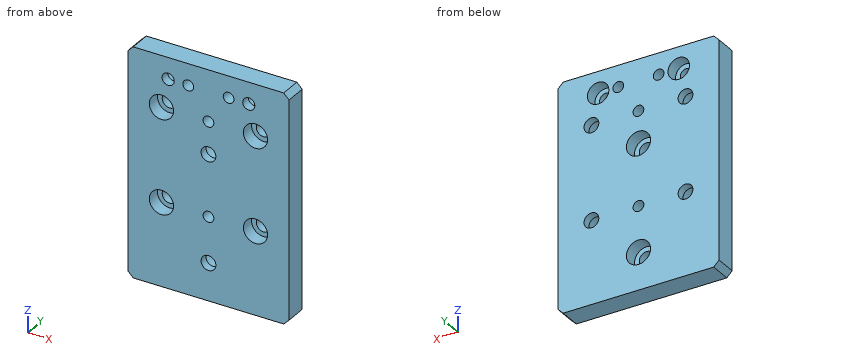
```python
from build123d import *

# Parameters (mm, degrees)
SKETCH_1_W                  = 60
SKETCH_1_H                  = 85
EXTRUDE_1_DEPTH             = 8
HOLE_WIZARD_1_D             = 5.5
HOLE_WIZARD_1_CBORE_D       = 9
HOLE_WIZARD_1_CBORE_DEPTH   = 5
HOLE_WIZARD_2_D             = 5.5
HOLE_WIZARD_2_DEPTH         = 12.4
HOLE_WIZARD_2_CBORE_D       = 9
HOLE_WIZARD_2_CBORE_DEPTH   = 5
HOLE_WIZARD_2_TIP           = 1.652366702
HOLE_WIZARD_1_2_D           = 4.5
HOLE_WIZARD_1_2_CBORE_D     = 8
HOLE_WIZARD_1_2_CBORE_DEPTH = 4.6
HOLE_WIZARD_4_0_4_1_D       = 4
CHAMFER_1_SIZE              = 2


with BuildPart() as part:
    # 草图1 → 凸台-拉伸1 (new body)
    with BuildSketch(Plane(origin=(0, 0, 0), x_dir=(1, 0, 0), z_dir=(0, 1, 0))):
        Rectangle(SKETCH_1_W, SKETCH_1_H)
    extrude(amount=EXTRUDE_1_DEPTH)

    # Hole Wizard 1 (through all)
    with Locations(Plane(origin=(0, 0, 0), x_dir=(-1, 0, 0), z_dir=(0, -1, 0))):
        with Locations((17.5, -23.45), (-17.5, -23.45), (17.5, 11.55), (-17.5, 11.55)):
            CounterBoreHole(HOLE_WIZARD_1_D / 2, HOLE_WIZARD_1_CBORE_D / 2, HOLE_WIZARD_1_CBORE_DEPTH)

    # 大小六角凹头盖螺钉柱孔2
    with Locations(Plane(origin=(0, 8, 0), x_dir=(1, 0, 0), z_dir=(0, 1, 0))):
        with Locations((0, 28.554479799), (0, -11.445520201)):
            CounterBoreHole(HOLE_WIZARD_2_D / 2, HOLE_WIZARD_2_CBORE_D / 2, HOLE_WIZARD_2_CBORE_DEPTH, depth=HOLE_WIZARD_2_DEPTH)
            with Locations((0, 0, -(HOLE_WIZARD_2_DEPTH + HOLE_WIZARD_2_TIP / 2))):  # 118° drill point
                Cone(0, HOLE_WIZARD_2_D / 2, HOLE_WIZARD_2_TIP, mode=Mode.SUBTRACT)

    # Hole Wizard 1 2 (through all)
    with Locations(Plane(origin=(0, 8, 0), x_dir=(1, 0, 0), z_dir=(0, 1, 0))):
        with Locations((-15, -34.5), (15, -34.5)):
            CounterBoreHole(HOLE_WIZARD_1_2_D / 2, HOLE_WIZARD_1_2_CBORE_D / 2, HOLE_WIZARD_1_2_CBORE_DEPTH)

    # Ø4.0 (4) 直径孔1 (through all)
    with Locations(Plane(origin=(0, 8, 0), x_dir=(1, 0, 0), z_dir=(0, 1, 0))):
        with Locations((-7.5, -34.5), (7.5, -34.5), (0, -23.45), (0, 11.55)):
            Hole(HOLE_WIZARD_4_0_4_1_D / 2)

    # 倒角1
    chamfer_1_edges = [part.edges().sort_by_distance(p)[0] for p in [
        (30, 4, 42.5),
        (-30, 4, 42.5),
        (-30, 4, -42.5),
        (30, 4, -42.5),
    ]]
    chamfer(chamfer_1_edges, length=CHAMFER_1_SIZE)


solid = part.part
```
Could you check a few things on this model? Use its own coordinates, in mm. Round coordinates to 2 decimals unless told otherwise and drop trailing zeros. Write each loop counter-clockwise with the first axis right and the second up, starting at its lowest first coordinate (ties: lowest second). Pieces come first, ordered by that corner, then holes. Notation, with made-up numbers: M 68.25,-6 L 104.25,-6 A15 ccw 104.25,11 Z; hole C 35,23 d11. An arc over 180 degrees is marked long. Answer in a Markdown table with one row per item. Add a question column.
Q1. Will these pins go through, and if not, where does the flat tip stop? pin 1 Ø4.5 at (x, z) = (-17.5, 23.45) entering from -Y; pin 2 Ø5 at (x, z) = (22, -27.5) entering from -Y; pin 3 Ø4 at (x, z) = (16, 33) entering from +Y; pin 4 Ø2.5 at (x, z) = (-2, -29.5) entering from +Y.
Q2. Imagine slicing it at B-B (z = 34.5). Please give me the cut outline in (x, y), then the cut area to 3 significant figures.
Q3. If I drill on line 1 (Z direction, x = 0, y = 5.25); line 2 (X direction, y = 2.6, z = 34.5); line 3 (X direction, y = 7, z = 23.45), over which ranges is the centre line in solid material (lowest first)? Write a range as from..to.
Q4. Imagine slicing it at A-A (x = -7.5). Please give me the cut outline in (y, z).
Q5. Imagine slicing it at C-C (z = -11.55). Please give me the cut outline in (x, y).
Q6. Imagine slicing it at D-D (x = 0). Please give me the cut outline in (y, z).
Values:
| question | item | result |
|---|---|---|
| 1 | pin 1 | through |
| 1 | pin 2 | y = 0 |
| 1 | pin 3 | y = 3.4 |
| 1 | pin 4 | y = 3 |
| 2 | outline | M -30,0 L -17.25,0 L -17.25,3.4 L -19,3.4 L -19,8 L -30,8 Z; M -12.75,0 L -9.5,0 L -9.5,8 L -11,8 L -11,3.4 L -12.75,3.4 Z; M -5.5,0 L 5.5,0 L 5.5,8 L -5.5,8 Z; M 9.5,0 L 12.75,0 L 12.75,3.4 L 11,3.4 L 11,8 L 9.5,8 Z; M 17.25,0 L 30,0 L 30,8 L 19,8 L 19,3.4 L 17.25,3.4 Z |
| 2 | area | 312 mm^2 |
| 3 | line 1 | -42.5..-33.05, -24.05..-13.55, -9.55..6.95, 15.95..21.45, 25.45..42.5 |
| 3 | line 2 | -30..-17.25, -12.75..-9.5, -5.5..5.5, 9.5..12.75, 17.25..30 |
| 3 | line 3 | -30..-20.25, -14.75..-2, 2..14.75, 20.25..30 |
| 4 | outline | M 0,-42.5 L 8,-42.5 L 8,32.5 L 0,32.5 Z; M 0,36.5 L 8,36.5 L 8,42.5 L 0,42.5 Z |
| 5 | outline | M -30,0 L -22,0 L -22,5 L -20.25,5 L -20.25,8 L -30,8 Z; M -14.75,5 L -13,5 L -13,0 L -2,0 L -2,8 L -14.75,8 Z; M 2,0 L 13,0 L 13,5 L 14.75,5 L 14.75,8 L 2,8 Z; M 20.25,5 L 22,5 L 22,0 L 30,0 L 30,8 L 20.25,8 Z |
| 6 | outline | M 0,-42.5 L 8,-42.5 L 8,-33.05 L 3,-33.05 L 3,-31.3 L 0,-31.3 Z; M 0,-25.8 L 3,-25.8 L 3,-24.05 L 8,-24.05 L 8,-13.55 L 0,-13.55 Z; M 0,-9.55 L 8,-9.55 L 8,6.95 L 3,6.95 L 3,8.7 L 0,8.7 Z; M 0,14.2 L 3,14.2 L 3,15.95 L 8,15.95 L 8,21.45 L 0,21.45 Z; M 0,25.45 L 8,25.45 L 8,42.5 L 0,42.5 Z |
